from build123d import *

# Parameters (mm, degrees)
BARREL_PROFILE_230_SKETCH_R  = 115
BARREL_BODY_230X2900_DEPTH   = 1450
END_TRIM_CUT_SKETCH_R        = 57.49999999999997
END_TRIM_CUT_DEPTH           = 1450
CLEVIS_EYE_PROFILE_SKETCH_W  = 365
CLEVIS_EYE_PROFILE_SKETCH_H  = 180.83378269641366
CLEVIS_EYE_PROFILE_CUT_DEPTH = 1450
EDGE_FILLET_R10_R            = 10


with BuildPart() as part:
    # Barrel Profile Ø230 Sketch → Barrel Body Ø230x2900 (new, symmetric)
    with BuildSketch(Plane.XY):
        Circle(BARREL_PROFILE_230_SKETCH_R)
    extrude(amount=BARREL_BODY_230X2900_DEPTH, both=True)

    # End Trim Cut Sketch → End Trim Cut (cut, symmetric)
    with BuildSketch(Plane(origin=(0, 0, 0), x_dir=(1, 0, 0), z_dir=(0, 1, 0))):
        with Locations(Location((0, 1305, 0), (0, 0, 270))):
            Circle(END_TRIM_CUT_SKETCH_R)
    extrude(amount=END_TRIM_CUT_DEPTH, both=True, mode=Mode.SUBTRACT)

    # Clevis Eye Profile Sketch → Clevis Eye Profile Cut (cut, symmetric)
    with BuildSketch(Plane(origin=(0, 0, 0), x_dir=(0, 0, -1), z_dir=(1, 0, 0))):
        with Locations((1267.5, -161.66689134820675)):
            Rectangle(CLEVIS_EYE_PROFILE_SKETCH_W, CLEVIS_EYE_PROFILE_SKETCH_H)
        with Locations((1267.5, 161.66689134820675)):
            Rectangle(CLEVIS_EYE_PROFILE_SKETCH_W, CLEVIS_EYE_PROFILE_SKETCH_H)
    extrude(amount=CLEVIS_EYE_PROFILE_CUT_DEPTH, both=True, mode=Mode.SUBTRACT)

    # Bore End Revolve Sketch → Bore End Revolved Cut (revolve, cut)
    with BuildSketch(Plane(origin=(0, 0, 0), x_dir=(1, 0, 0), z_dir=(0, 1, 0)), mode=Mode.PRIVATE) as bore_end_revolved_cut_sk:
        with BuildLine():
            Line((0, 1537.1393692003157), (209.05243850437193, 1537.1393692003157))
            Line((209.05243850437193, 1537.1393692003157), (209.05243850437193, 1305))
            Line((209.05243850437193, 1305), (115, 1305))
            ThreePointArc((115, 1305), (81.31727983645297, 1386.317279836453), (0, 1420))
            Line((0, 1420), (0, 1537.1393692003157))
        make_face()
    revolve(bore_end_revolved_cut_sk.sketch.rotate(Axis((0, 0, -1420), (0, 0, -1)), 218.284391292), axis=Axis((0, 0, -1420), (0, 0, -1)), mode=Mode.SUBTRACT)

    # Eye End Revolve Sketch → Eye End Revolved Cut (revolve, cut)
    with BuildSketch(Plane(origin=(0, 0, 0), x_dir=(1, 0, 0), z_dir=(0, 1, 0))):
        Polygon((0, -1450), (-6.94e-15, 1034.9999999999995), (81, 1035), (81, -1420), (66, -1420), (66, -1450), align=None)
    revolve(axis=Axis((0, 0, 1450), (0, 0, -1)), mode=Mode.SUBTRACT)

    # Edge Fillet R10
    edge_fillet_r10_edges = [part.edges().sort_by_distance(p)[0] for p in [
        (-115, 1.408e-14, 1450),
    ]]
    fillet(edge_fillet_r10_edges, radius=EDGE_FILLET_R10_R)


solid = part.part
Model file for the job. Use its own axes, mm. A direction names the side the tool comes from. Coordinates: 2 decimals unless noted, no trailing zeros. Order: outer loops, then holes, each group sorted by start corner. A loop starts at its lowest first (then second) coordinate and runs counter-clockwise, first axis right, second up. Notation, with made-up numbers: M 67.25,37 L 107.25,37 A6 cw 107.25,48 Z; hole C -27.5,72.5 d11. An arc over 180 degrees is marked long. Return JSON: item names as keys, results as strings.
1. Tool access for faces 4 (the face through (60.967, 25.278, 1435.21)), 5 (the face through (-1, -71.25, -1203)), 6 (the face through (-66.4, -0.4, 1420)), 7 (the face through (53.065, -102.025, 86.715)): list every direction of +Z, -Z, +X, -X, +Y, -Y with a clear straight run to the whole face (end or side of a thin tool).
Ans:
{"face 4": "+Z", "face 5": "-Z, +X, -X, -Y", "face 6": "none", "face 7": "+Z, -Z"}
2. Saw through at D-D (z = -150.5). Give the cut face in (x, y).
Ans:
{"outline": "C 0,0 d230; hole C 0,0 d162"}
3. Saw through at C-C (z = -1171). Give the cut face in (x, y).
Ans:
{"outline": "M -90.27,-71.25 L 90.27,-71.25 A115 ccw 90.27,71.25 L -90.27,71.25 A115 ccw Z"}
4. Saw through at A-A (y = 0). Give the cut face in (x, z), and give its area (3 significant figures).
Ans:
{"outline": "M -115,-1305 A115 ccw 115,-1305 L 115,1440 A10 ccw 105,1450 L 66,1450 L 66,1420 L 81,1420 L 81,-1035 L -81,-1035 L -81,1420 L -66,1420 L -66,1450 L -105,1450 A10 ccw -115,1440 Z; hole C 0,-1305 d115", "area": "242,000 mm^2"}
5. Flat gauge pins, fed straight in: pin 1 (2 mm diameter, centred on x = -2.5, z = -346, fed in from -Y); pin 2 (1.5 mm diameter, centred on x = 73.5, z = -26, fed in from -Y); pin 3 (2 mm diameter, centred on x = 26.5, z = 1047.5, fed in from -Y). Where does each tip first touch, or does it go through?
Ans:
{"pin 1": "y = -114.99", "pin 2": "y = -89.06", "pin 3": "y = -112.14"}
6. Drill centre lines: probe 1 along Y at (x, z) = (-46.5, -208); probe 2 along Y at (x, z) = (-3.5, 540.5); probe 3 along X at (y, z) = (0, -490.5). Where is each one in solid material? Low to high.
Ans:
{"probe 1": "-105.18 to -66.32, 66.32 to 105.18", "probe 2": "-114.95 to -80.92, 80.92 to 114.95", "probe 3": "-115 to -81, 81 to 115"}
7. Saw through at B-B (x = 0). Give the cut face in (y, z).
Ans:
{"outline": "M -115,-1085 L -71.25,-1085 L -71.25,-1247.5 L 71.25,-1247.5 L 71.25,-1085 L 115,-1085 L 115,1440 A10 ccw 105,1450 L 66,1450 L 66,1420 L 81,1420 L 81,-1035 L -81,-1035 L -81,1420 L -66,1420 L -66,1450 L -105,1450 A10 ccw -115,1440 Z; M -71.25,-1395.27 A115 ccw 71.25,-1395.27 L 71.25,-1362.5 L -71.25,-1362.5 Z"}
8. Pull direction Z, two halves, no side cores. Call faces 1 (the face through (1, 88, -1085)), 2 (the face through (2.528, 0.998, -1362.444)), 3 (the face through (1, 71.25, -1203)): +Z half, -Z half, draft (parallel to the pull), parting line (faces both ways), or undercut.
Ans:
{"face 1": "-Z half", "face 2": "undercut", "face 3": "draft"}
